Check sheet for the drawn part. Datum: minimum x, y, z corner. Units: mm. A direction names the side the tool comes from. Give positions to 0.01 mm unless a question says otherwise; leave off trailing zeros. Loops run counter-clockwise (first coordinate to the right, second up) from the corner with the lowest first, then second, coordinate; pieces in that order, holes last. Notation, with made-up numbers: (21.25, 63) - (39.25, 63) arc R21 ccw to (39.25, 86) - close; hole circle Ø8 at (4.5, 34.25). An arc over 180 degrees is marked (long way). Use a Markdown table: item, result. Add a question column.
1. Material ranges on L1, parallel to Y at x = 4.5, z = 7; L2, parallel to Y at x = 3.5, z = 7; L3, parallel to Z at x = 0.5, y = 11.5, recorded low to high.
2. Cross-section at C-C on x = 8. Enter the section's corners in (y, z).
3. Depth check by flat-ended pin: P1, Ø6.5, axis at y = 13.5, z = 7, coming from the +X side. Enter the tip coordinate at first touch or a pass-through.
4. Draft check along Z on the marked faces 1, 2 and 3. Enter one of: pulls with the +Z half, pulls with the -Z half, needs draft (parallel to the pull), parting line crosses it, or undercut.
5. Cross-section at A-A on y = 24. Enter the section's corners in (x, z).
6. Cross-section at B-B on z = 7. Enter the section's corners in (x, y).
7. Cross-section at D-D on y = 10. Enter the section's corners in (x, z).
8. Set-up check for the marked faces 4, 5 and 6: record each of +Z, -Z, +X, -X, +Y, -Y from which the full face is reachable in a straight line by a thin tool's end or side.
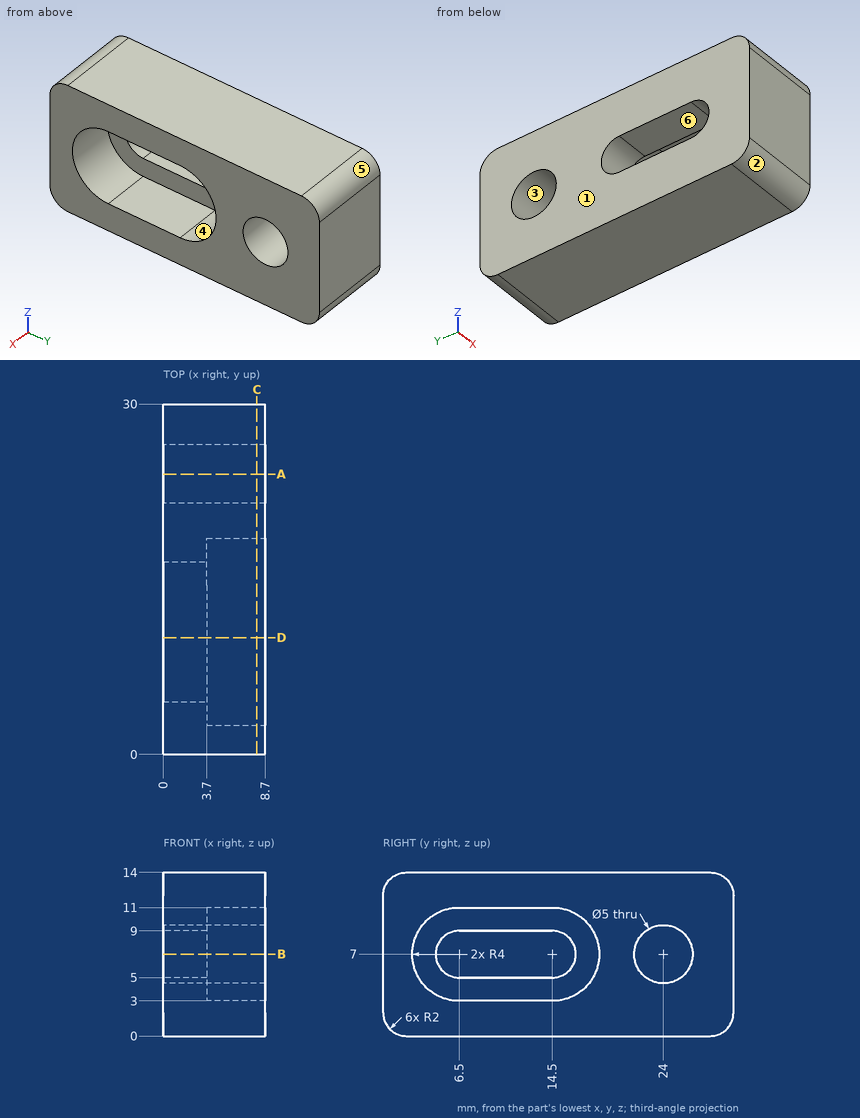
Values found:
| question | item | result |
|---|---|---|
| 1 | L1 | y = 0 to 2.5, 18.5 to 21.5, 26.5 to 30 |
| 1 | L2 | y = 0 to 4.5, 16.5 to 21.5, 26.5 to 30 |
| 1 | L3 | z = 0 to 5, 9 to 14 |
| 2 | outline | (0, 2) arc R2 ccw to (2, 0) - (28, 0) arc R2 ccw to (30, 2) - (30, 12) arc R2 ccw to (28, 14) - (2, 14) arc R2 ccw to (0, 12) - close; hole (6.5, 3) - (14.5, 3) arc R4 ccw to (14.5, 11) - (6.5, 11) arc R4 ccw to start; hole circle Ø5 at (24, 7) |
| 3 | P1 | stops at x = 3.7 |
| 4 | face 1 | needs draft |
| 4 | face 2 | pulls with the -Z half |
| 4 | face 3 | undercut |
| 5 | outline | (0, 0) - (8.7, 0) - (8.7, 4.5) - (0, 4.5) - close; (0, 9.5) - (8.7, 9.5) - (8.7, 14) - (0, 14) - close |
| 6 | outline | (0, 0) - (8.7, 0) - (8.7, 2.5) - (3.7, 2.5) - (3.7, 4.5) - (0, 4.5) - close; (0, 16.5) - (3.7, 16.5) - (3.7, 18.5) - (8.7, 18.5) - (8.7, 21.5) - (0, 21.5) - close; (0, 26.5) - (8.7, 26.5) - (8.7, 30) - (0, 30) - close |
| 7 | outline | (0, 0) - (8.7, 0) - (8.7, 3) - (3.7, 3) - (3.7, 5) - (0, 5) - close; (0, 9) - (3.7, 9) - (3.7, 11) - (8.7, 11) - (8.7, 14) - (0, 14) - close |
| 8 | face 4 | +X |
| 8 | face 5 | +Z, +X, -X, +Y |
| 8 | face 6 | +X, -X |
